from build123d import *

# Parameters (mm, degrees)
SKETCH_1_W                  = 450
SKETCH_1_H                  = 65
EXTRUDE_1_DEPTH             = 15
CHAMFER_1_SIZE              = 2
SKETCH_2_R                  = 10
CUT_EXTRUDE_1_DEPTH         = 30
CUT_EXTRUDE_2_DEPTH         = 30
SKETCH_4_R                  = 21
CUT_EXTRUDE_3_DEPTH         = 12
SKETCH_5_R                  = 18
CUT_EXTRUDE_4_DEPTH         = 229.046596116
HOLE_WIZARD_2_D             = 6.6
HOLE_WIZARD_2_DEPTH         = 31.5
HOLE_WIZARD_2_CBORE_D       = 11
HOLE_WIZARD_2_CBORE_DEPTH   = 6.8
HOLE_WIZARD_M6_1_D          = 5
HOLE_WIZARD_2_2_D           = 9
HOLE_WIZARD_2_2_CBORE_D     = 15
HOLE_WIZARD_2_2_CBORE_DEPTH = 55
HOLE_WIZARD_M5_1_D          = 4.2
HOLE_WIZARD_M5_1_DEPTH      = 12.4
HOLE_WIZARD_M5_1_TIP        = 1.2618073
SKETCH_15_W                 = 237.437546179
SKETCH_15_H                 = 159.818796437
CUT_EXTRUDE_6_DEPTH         = 230.306018238


with BuildPart() as part:
    # 草图1 → 凸台-拉伸1 (new, symmetric)
    with BuildSketch(Plane(origin=(0, 0, 0), x_dir=(1, 0, 0), z_dir=(0, 1, 0))):
        Rectangle(SKETCH_1_W, SKETCH_1_H)
    extrude(amount=EXTRUDE_1_DEPTH, both=True)

    # 倒角1
    chamfer_1_edges = [part.edges().sort_by_distance(p)[0] for p in [
        (225, 0, 32.5),
        (-225, 0, 32.5),
    ]]
    chamfer(chamfer_1_edges, length=CHAMFER_1_SIZE)

    # 草图2 → 切除-拉伸1 (cut)
    with BuildSketch(Plane(origin=(0, 15, 0), x_dir=(1, 0, 0), z_dir=(0, 1, 0))):
        with Locations(Location((-200, 0, 0), (0, 0, 270))):
            Circle(SKETCH_2_R)
        with Locations(Location((200, 0, 0), (0, 0, 90))):
            Circle(SKETCH_2_R)
    extrude(amount=-CUT_EXTRUDE_1_DEPTH, mode=Mode.SUBTRACT)

    # 草图3 → 切除-拉伸2 (cut)
    with BuildSketch(Plane(origin=(0, 15, 0), x_dir=(1, 0, 0), z_dir=(0, 1, 0))):
        with BuildLine():
            Line((-225, 1), (-182, 1))
            ThreePointArc((-182, 1), (-181, 0), (-182, -1))
            Line((-182, -1), (-225, -1))
            ThreePointArc((-225, -1), (-226, 0), (-225, 1))
        make_face()
        with BuildLine():
            Line((225, 1), (182, 1))
            ThreePointArc((182, 1), (181, 0), (182, -1))
            Line((182, -1), (225, -1))
            ThreePointArc((225, -1), (226, 0), (225, 1))
        make_face()
    extrude(amount=-CUT_EXTRUDE_2_DEPTH, mode=Mode.SUBTRACT)

    # 草图4 → 切除-拉伸3 (cut)
    with BuildSketch(Plane(origin=(0, -15, 0), x_dir=(1, 0, 0), z_dir=(0, 1, 0))):
        with Locations(Location((0, -7.5, 0), (0, 0, 270))):
            Circle(SKETCH_4_R)
    extrude(amount=CUT_EXTRUDE_3_DEPTH, mode=Mode.SUBTRACT)

    # 草图5 → 切除-拉伸4 (cut, through all)
    with BuildSketch(Plane(origin=(0, -3, 0), x_dir=(-1, 0, 0), z_dir=(0, -1, 0))):
        with Locations(Location((0, -7.5, 0), (0, 0, 90))):
            Circle(SKETCH_5_R)
    extrude(amount=-CUT_EXTRUDE_4_DEPTH, mode=Mode.SUBTRACT)

    # Hole Wizard 2
    with Locations(Plane.XY.offset(32.5)):
        with Locations((215, -7.5), (215, 7.5), (-215, 7.5), (-215, -7.5)):
            CounterBoreHole(HOLE_WIZARD_2_D / 2, HOLE_WIZARD_2_CBORE_D / 2, HOLE_WIZARD_2_CBORE_DEPTH, depth=HOLE_WIZARD_2_DEPTH)

    # M6 螺纹孔1 (through all)
    with Locations(Plane.XY.offset(-1)):
        with Locations((215, -7.5), (215, 7.5), (-215, -7.5), (-215, 7.5)):
            Hole(HOLE_WIZARD_M6_1_D / 2)

    # Hole Wizard 2 2 (through all)
    with Locations(Plane.XY.offset(32.5)):
        with Locations((150, 0), (30, 0), (-30, 0), (-150, 0)):
            CounterBoreHole(HOLE_WIZARD_2_2_D / 2, HOLE_WIZARD_2_2_CBORE_D / 2, HOLE_WIZARD_2_2_CBORE_DEPTH)

    # M5 螺纹孔1
    with Locations(Plane(origin=(0, -15, 0), x_dir=(-1, 0, 0), z_dir=(0, -1, 0))):
        with Locations((-17.324116139, 9.824116139), (17.324116139, 9.824116139), (17.324116139, -24.824116139), (-17.324116139, -24.824116139)):
            Hole(HOLE_WIZARD_M5_1_D / 2, depth=HOLE_WIZARD_M5_1_DEPTH)
            with Locations((0, 0, -(HOLE_WIZARD_M5_1_DEPTH + HOLE_WIZARD_M5_1_TIP / 2))):  # 118° drill point
                Cone(0, HOLE_WIZARD_M5_1_D / 2, HOLE_WIZARD_M5_1_TIP, mode=Mode.SUBTRACT)

    # 草图15 → 切除-拉伸6 (cut, through all)
    with BuildSketch(Plane.XZ.offset(15)):
        with Locations((158.71877309, 13.745723836)):
            Rectangle(SKETCH_15_W, SKETCH_15_H)
        with Locations((-158.71877309, 13.745723836)):
            Rectangle(SKETCH_15_W, SKETCH_15_H)
    extrude(amount=-CUT_EXTRUDE_6_DEPTH, mode=Mode.SUBTRACT)


solid = part.part
The listing builds one solid part. Answer for the finished solid, in the listing's coordinates (mm). A direction names the side the tool comes from. Round coordinates to 2 decimals unless told otherwise and drop trailing zeros. Order: outer loops, then holes, each group sorted by start corner. A loop starts at its lowest first (then second) coordinate and runs counter-clockwise, first axis right, second up. Notation, with made-up numbers: (-22.75, 30.5) -> (22.25, 30.5) arc R26 cw to (22.25, 52.5) -> close; hole circle Ø2 at (16.5, 60). An arc over 180 degrees is marked (long way). Write each question's results on one line, items separated by ' | '. Start each with the question number.
Q1. Which of the six approach directions +Z, -Z, +X, -X, +Y, -Y give full straight-line access (tool end or side, diameter ignored) to faces 1 (the flat face through (35, 0, -22.5)), 2 (the flat face through (6, -3, 25)), 3 (the flat face through (-1, 0, 32.5))?
Q2. Find section D-D (y = 6). Determine the outline of the cut face in (x, z).
Q3. Each of these flat-tipped pins is pushed along its axis until it touches: pin 1 (2.5 mm diameter, centred on x = -17.32, z = -9.82, fed in from -Y); pin 2 (14.5 mm diameter, centred on x = -30, y = 0, fed in from +Z); pin 3 (21 mm diameter, centred on x = -8.5, z = 6, fed in from -Y). Where does it stop, or does it pass through?
Q4. The mould has two halves that part along X. Classify faces 4 (the flat face through (-1, -15, -15)), 5 (the flat face through (-40, 0, 0)), 6 (the conical face through (17.37, -1.56, -10.19)): pulls with the +X half, pulls with the -X half, needs draft (parallel to the pull), parting line crosses it, or undercut.
Q5. Find section B-B (y = 0). Determine the outline of the cut face in (x, z).
Q6. Straight lines are drawn through the part: probe 1 along X at (y, z) = (1.75, -7); probe 2 along X at (y, z) = (9.5, 7.5); probe 3 along Y at (x, z) = (-30, 0.5). For each, find the intervals that lie inside material, in ascending order. Write a range as from..to.
Q7. Find section A-A (z = 7.5). Determine the outline of the cut face in (x, y).
Q8. Find section C-C (x = 30). Determine the outline of the cut face in (y, z).
Worked answers:
1) face 1: +Z | face 2: -Y | face 3: +Z, +X, -X, +Y, -Y
2) outline: (-40, -32.5) -> (40, -32.5) -> (40, 32.5) -> (34.5, 32.5) -> (34.5, -22.5) -> (25.5, -22.5) -> (25.5, 32.5) -> (-25.5, 32.5) -> (-25.5, -22.5) -> (-34.5, -22.5) -> (-34.5, 32.5) -> (-40, 32.5) -> close; hole circle Ø36 at (0, 7.5)
3) pin 1: stops at y = -2.09 | pin 2: stops at z = -22.5 | pin 3: stops at y = -3
4) face 4: needs draft | face 5: pulls with the -X half | face 6: undercut
5) outline: (-40, -32.5) -> (-34.5, -32.5) -> (-34.5, -22.5) -> (-37.5, -22.5) -> (-37.5, 32.5) -> (-40, 32.5) -> close; (-25.5, -32.5) -> (25.5, -32.5) -> (25.5, -22.5) -> (22.5, -22.5) -> (22.5, 32.5) -> (-22.5, 32.5) -> (-22.5, -22.5) -> (-25.5, -22.5) -> close; (34.5, -32.5) -> (40, -32.5) -> (40, 32.5) -> (37.5, 32.5) -> (37.5, -22.5) -> (34.5, -22.5) -> close; hole circle Ø36 at (0, 7.5)
6) probe 1: x = -40..-37.29, -22.71..-10.67, 10.67..22.71, 37.29..40 | probe 2: x = -40..-18, 18..40 | probe 3: y = -15..-7.5, 7.5..15
7) outline: (-40, -15) -> (-21, -15) -> (-21, -3) -> (-18, -3) -> (-18, 15) -> (-40, 15) -> close; (18, -3) -> (21, -3) -> (21, -15) -> (40, -15) -> (40, 15) -> (18, 15) -> close; hole circle Ø15 at (-30, 0); hole circle Ø15 at (30, 0)
8) outline: (-15, -32.5) -> (-4.5, -32.5) -> (-4.5, -22.5) -> (-7.5, -22.5) -> (-7.5, 32.5) -> (-15, 32.5) -> close; (4.5, -32.5) -> (15, -32.5) -> (15, 32.5) -> (7.5, 32.5) -> (7.5, -22.5) -> (4.5, -22.5) -> close
